```python
from build123d import *

# Parameters (mm, degrees)
SKETCH1_W           = 70
SKETCH1_H           = 50
BOSS_EXTRUDE1_DEPTH = 40
SKETCH2_R           = 5
CUT_EXTRUDE1_DEPTH  = 95.868329805
SKETCH3_R           = 6
CUT_EXTRUDE2_DEPTH  = 35
SKETCH4_R           = 10.5
CUT_EXTRUDE3_DEPTH  = 7
FILLET1_R           = 3


with BuildPart() as part:
    # Sketch1 → Boss-Extrude1 (new body)
    with BuildSketch(Plane(origin=(0, 0, 0), x_dir=(1, 0, 0), z_dir=(0, 1, 0))):
        with Locations((35, 25)):
            Rectangle(SKETCH1_W, SKETCH1_H)
    extrude(amount=BOSS_EXTRUDE1_DEPTH)

    # Sketch2 → Cut-Extrude1 (cut, through all)
    with BuildSketch(Plane(origin=(70, 0, 0), x_dir=(0, 0, -1), z_dir=(1, 0, 0))):
        with Locations((40, 25)):
            Circle(SKETCH2_R)
        with Locations((10, 25)):
            Circle(SKETCH2_R)
    extrude(amount=-CUT_EXTRUDE1_DEPTH, mode=Mode.SUBTRACT)

    # Sketch3 → Cut-Extrude2 (cut)
    with BuildSketch(Plane.XZ):
        with Locations(Location((60, -25, 0), (0, 0, 270))):
            Circle(SKETCH3_R)
    extrude(amount=-CUT_EXTRUDE2_DEPTH, mode=Mode.SUBTRACT)

    # Sketch4 → Cut-Extrude3 (cut)
    with BuildSketch(Plane.XZ):
        with Locations(Location((15, -25, 0), (0, 0, 270))):
            Circle(SKETCH4_R)
    extrude(amount=-CUT_EXTRUDE3_DEPTH, mode=Mode.SUBTRACT)

    # Fillet1
    fillet1_edges = [part.edges().sort_by_distance(p)[0] for p in [
        (70, 40, -25),
        (35, 40, -50),
        (0, 40, -25),
        (35, 0, -50),
        (70, 0, -25),
        (35, 0, 0),
        (0, 0, -25),
        (35, 40, 0),
        (0, 20, -50),
        (70, 20, -50),
        (70, 20, 0),
        (0, 20, 0),
    ]]
    fillet(fillet1_edges, radius=FILLET1_R)


solid = part.part
```
Geometry: final body of the model. Coordinates: model frame, mm. Coordinates: 2 decimals unless noted, no trailing zeros. Order: outer loops, then holes, each group sorted by start corner. A loop starts at its lowest first (then second) coordinate and runs counter-clockwise, first axis right, second up. Notation, with made-up numbers: (80, 81.5) -> (134, 81.5) arc R21 cw to (134, 100.5) -> close; hole circle Ø5 at (17, -40). An arc over 180 degrees is marked (long way). Use CSV: the item, a comma, the result in double quotes.
1) Mould query, pull axis X, two halves, no side actions, for faces 1 (the flat face through (35, 20, 0)), 2 (the flat face through (15, 7, -25)), 3 (the cylindrical face through (0.86, 20.24, -49.1)), 4 (the cylindrical face through (69.1, 20.24, -0.86)). Classes: +X half, -X half, draft (parallel to the pull), parting line (faces both ways), or undercut.
Findings:
face 1,"draft"
face 2,"undercut"
face 3,"-X half"
face 4,"+X half"
2) Section B-B on z = -10. Output: boundary loops of the cut face in (x, y), then the cut area to 3 significant figures.
Findings:
outline,"(0, 3) arc R3 ccw to (3, 0) -> (67, 0) arc R3 ccw to (70, 3) -> (70, 20) -> (0, 20) -> close; (0, 30) -> (70, 30) -> (70, 37) arc R3 ccw to (67, 40) -> (3, 40) arc R3 ccw to (0, 37) -> close"
area,"2,090 mm^2"
3) Section A-A on y = 25. Output: boundary loops of the cut face in (x, z), then the cut area to 3 significant figures.
Findings:
outline,"(0, -47) arc R3 ccw to (3, -50) -> (67, -50) arc R3 ccw to (70, -47) -> (70, -45) -> (0, -45) -> close; (0, -35) -> (70, -35) -> (70, -15) -> (0, -15) -> close; (0, -5) -> (70, -5) -> (70, -3) arc R3 ccw to (67, 0) -> (3, 0) arc R3 ccw to (0, -3) -> close; hole circle Ø12 at (60, -25)"
area,"1,980 mm^2"
4) Section C-C on x = 60. Output: boundary loops of the cut face in (y, z).
Findings:
outline,"(0, -47) arc R3 ccw to (3, -50) -> (37, -50) arc R3 ccw to (40, -47) -> (40, -3) arc R3 ccw to (37, 0) -> (3, 0) arc R3 ccw to (0, -3) -> (0, -19) -> (35, -19) -> (35, -31) -> (0, -31) -> close; hole circle Ø10 at (25, -40); hole circle Ø10 at (25, -10)"
5) Pin query (flat end, axial travel): pin 1 Ø6.5 at (x, z) = (18.5, -20) entering from -Y; pin 2 Ø3.5 at (x, z) = (59, -25) entering from -Y. Return the tip coordinate at first contact, or that it passes through.
Findings:
pin 1,"stops at y = 7"
pin 2,"stops at y = 35"
6) Section D-D on y = 31. Output: boundary loops of the cut face in (x, z).
Findings:
outline,"(0, -47) arc R3 ccw to (3, -50) -> (67, -50) arc R3 ccw to (70, -47) -> (70, -3) arc R3 ccw to (67, 0) -> (3, 0) arc R3 ccw to (0, -3) -> close; hole circle Ø12 at (60, -25)"
7) Line query: line 1 (X direction, y = 25.5, z = -25); line 2 (Y direction, x = 30, z = -40); line 3 (Z direction, x = 33.5, y = 20.5). Output: solid intervals per line, ascending.
Findings:
line 1,"x = 0 to 54, 66 to 70"
line 2,"y = 0 to 20, 30 to 40"
line 3,"z = -50 to -42.18, -37.82 to -12.18, -7.82 to 0"
